from build123d import *

# Parameters (mm, degrees)
EXTRUDE_387_DEPTH = 7.5
FILLET_1310_R     = 0.6


with BuildPart() as part:
    # 草图1 → Extrude 387 (new body)
    with BuildSketch(Plane(origin=(0, 0, 0), x_dir=(0, 0, -1), z_dir=(1, 0, 0))):
        Polygon((9, 5.196152423), (9, -5.196152423), (0, -10.392304845), (-9, -5.196152423), (-9, 5.196152423), (0, 10.392304845), align=None)
    extrude(amount=EXTRUDE_387_DEPTH)

    # 草图2 → 凸台-旋转1 (revolve)
    with BuildSketch(Plane.XY, mode=Mode.PRIVATE) as revolve_1_sk:
        Polygon((0, 0), (67.5, 0), (67.5, 4.4845), (67.5, 6), (37.5, 6), (0, 6), align=None)
    revolve(revolve_1_sk.sketch.rotate(Axis((0, 0, 0), (1, 0, 0)), 90), axis=Axis((0, 0, 0), (1, 0, 0)))

    # 草图3 → 切除-旋转1 (revolve, cut)
    with BuildSketch(Plane.XY):
        Polygon((0, 9), (3.690598923, 15.392304845), (3.690598923, 20.392304845), (-10, 20.392304845), (-10, 9), align=None)
    revolve(axis=Axis((0, 0, 0), (1, 0, 0)), mode=Mode.SUBTRACT)

    # 草图4 → 切除-旋转3 (revolve, cut)
    with BuildSketch(Plane.XY, mode=Mode.PRIVATE) as cut_revolve_3_sk:
        Polygon((7.5, 8.315), (6.9, 8.661410162), (6.9, 10.392304845), (7.5, 10.392304845), align=None)
    revolve(cut_revolve_3_sk.sketch.rotate(Axis((0, 0, 0), (1, 0, 0)), 90), axis=Axis((0, 0, 0), (1, 0, 0)), mode=Mode.SUBTRACT)

    # Fillet 1310
    fillet_1310_edges = [part.edges().sort_by_distance(p)[0] for p in [
        (7.5, 0, -6),
    ]]
    fillet(fillet_1310_edges, radius=FILLET_1310_R)


solid = part.part
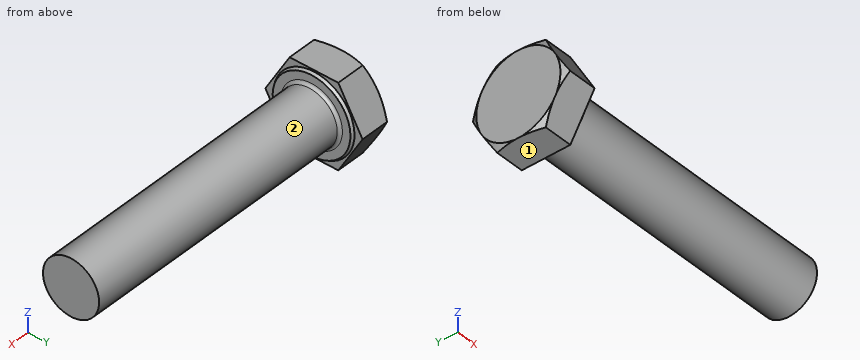
For this review, take the finished solid that the model builds, in its own axes (mm). Face numbers are marked on the shaded views. A direction names the side the tool comes from. Give positions to 0.01 mm unless a question says otherwise; leave off trailing zeros. Loops run counter-clockwise (first coordinate to the right, second up) from the corner with the lowest first, then second, coordinate; pieces in that order, holes last.
Item 1: Tool access review of the marked faces 1 and 2: name each direction out of +Z, -Z, +X, -X, +Y, -Y from which nothing blocks a thin tool from reaching the whole face with its end or side.
Item 2: Insertion check: pin 1 (8 mm diameter, centred on x = 52.5, z = 5, fed in from -Y); pin 2 (1 mm diameter, centred on x = 24, z = -2, fed in from -Y); pin 3 (2 mm diameter, centred on x = 23, z = -4.5, fed in from +Y). Each pin has a flat end and moves straight along its axis. Give the tip position at first contact, or say it passes through.
Item 3: For line 1 along X through (y, z) = (-7.25, -1.5); line 2 along Y through (x, z) = (11, -4); line 3 along Z through (x, y) = (29.5, 2.5), list the stretches that pass through material, from the lowest coordinate up.
Item 4: Take a section at A-A, the plane x = 57.5. State the section outline as (y, z) points, and give its area (3 significant figures).
Calculated:
1. face 1: -Z, +X, -X, +Y, -Y
1. face 2: +X
2. pin 1: stops at y = -5.92
2. pin 2: stops at y = -5.81
2. pin 3: stops at y = 4.87
3. line 1: x = 0 to 7.5
3. line 2: y = -4.47 to 4.47
3. line 3: z = -5.45 to 5.45
4. outline: circle Ø12 at (0, 0)
4. area: 113 mm2
